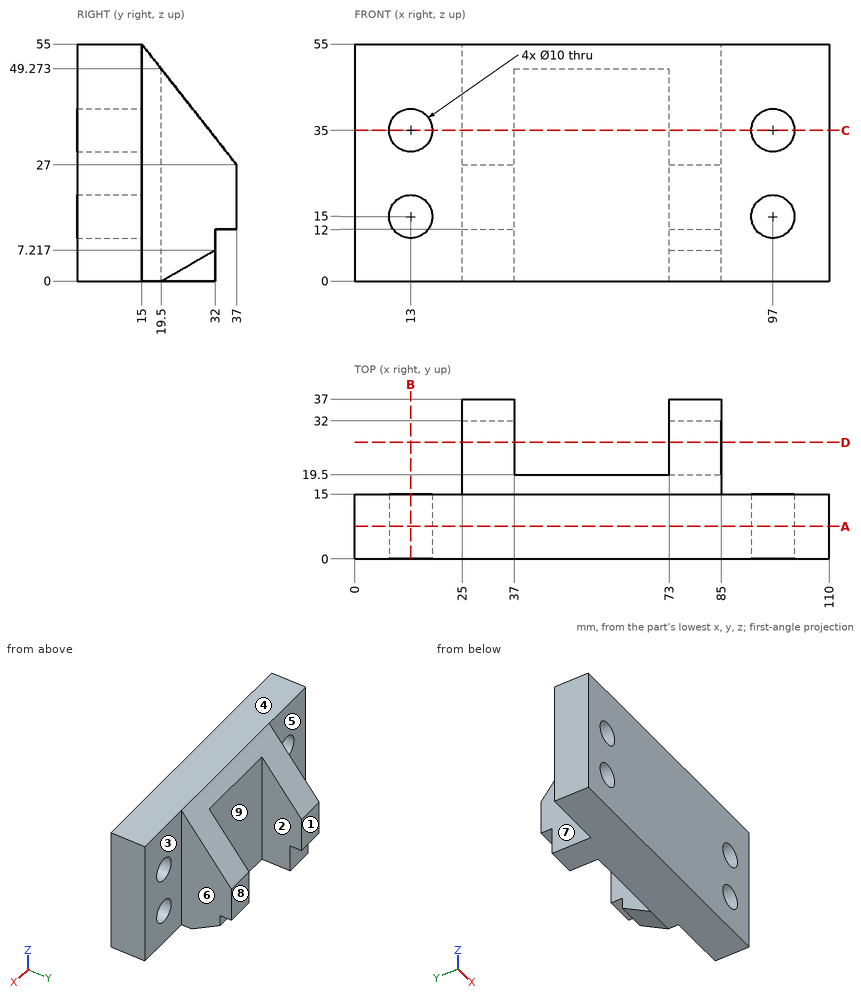
Part print with two shaded views. Sizes in mm from the minimum x, y, z corner. A direction names the side the tool comes from. Coordinates: 2 decimals unless noted, no trailing zeros. Write each loop counter-clockwise with the first axis right and the second up, starting at its lowest first coordinate (ties: lowest second). Pieces come first, ordered by that corner, then holes.
(1) Drill centre lines: line 1 (Z direction, x = 97, y = 7.75); line 2 (X direction, y = 4, z = 15); line 3 (X direction, y = 26, z = 18.5). Where is each one in solid material? Low to high.
(2) Cut at D-D on y = 27. List the corners of the cut face in (x, z).
(3) Cut at C-C on z = 35. List the corners of the cut face in (x, y), and give its area (3 significant figures).
(4) Cut at B-B on x = 13. List the corners of the cut face in (y, z).
(5) Mould opens along X. For the marked faces 6, 7, 8 and 9 say: pulls with the +X half, pulls with the -X half, needs draft (parallel to the pull), parting line crosses it, or undercut.
(6) Pin check, flat tips, straight feed: pin 1 Ø8 at (y, z) = (20, 35) entering from +X; pin 2 Ø5.5 at (x, z) = (76.5, 9) entering from +Y; pin 3 Ø7.5 at (x, z) = (95.5, 25.5) entering from +Y. Stop position of each tip, or through.
(7) Cut at A-A on y = 7.5. List the corners of the cut face in (x, z), and give its area (3 significant figures).
(8) 3-axis set-ups, long thin cutter, end or side, ignore diameter. For the marked faces 1, 2, 3, 4 and 5: which of +Z, -Z, +X, -X, +Y, -Y reach the whole face in a straight line?
Working result:
1. line 1: z = 0 to 10, 20 to 30, 40 to 55
1. line 2: x = 0 to 8, 18 to 92, 102 to 110
1. line 3: x = 25 to 37, 73 to 85
2. outline: (25, 0) - (37, 0) - (37, 39.73) - (25, 39.73) - close; (73, 4.33) - (85, 4.33) - (85, 39.73) - (73, 39.73) - close
3. outline: (0, 0) - (8, 0) - (8, 15) - (0, 15) - close; (18, 0) - (92, 0) - (92, 15) - (85, 15) - (85, 30.71) - (73, 30.71) - (73, 19.5) - (37, 19.5) - (37, 30.71) - (25, 30.71) - (25, 15) - (18, 15) - close; (102, 0) - (110, 0) - (110, 15) - (102, 15) - close
3. area: 1,890 mm2
4. outline: (0, 0) - (15, 0) - (15, 10) - (0, 10) - close; (0, 20) - (15, 20) - (15, 30) - (0, 30) - close; (0, 40) - (15, 40) - (15, 55) - (0, 55) - close
5. face 6: pulls with the +X half
5. face 7: pulls with the -X half
5. face 8: needs draft
5. face 9: undercut
6. pin 1: stops at x = 85
6. pin 2: stops at y = 32
6. pin 3: stops at y = 15
7. outline: (0, 0) - (110, 0) - (110, 55) - (0, 55) - close; hole circle Ø10 at (13, 15); hole circle Ø10 at (13, 35); hole circle Ø10 at (97, 15); hole circle Ø10 at (97, 35)
7. area: 5,740 mm2
8. face 1: +Z, -Z, +X, -X, +Y
8. face 2: +Z, -Z, +Y
8. face 3: +Z, -Z, +X, +Y
8. face 4: +Z, +X, -X, +Y, -Y
8. face 5: +Z, -Z, -X, +Y
